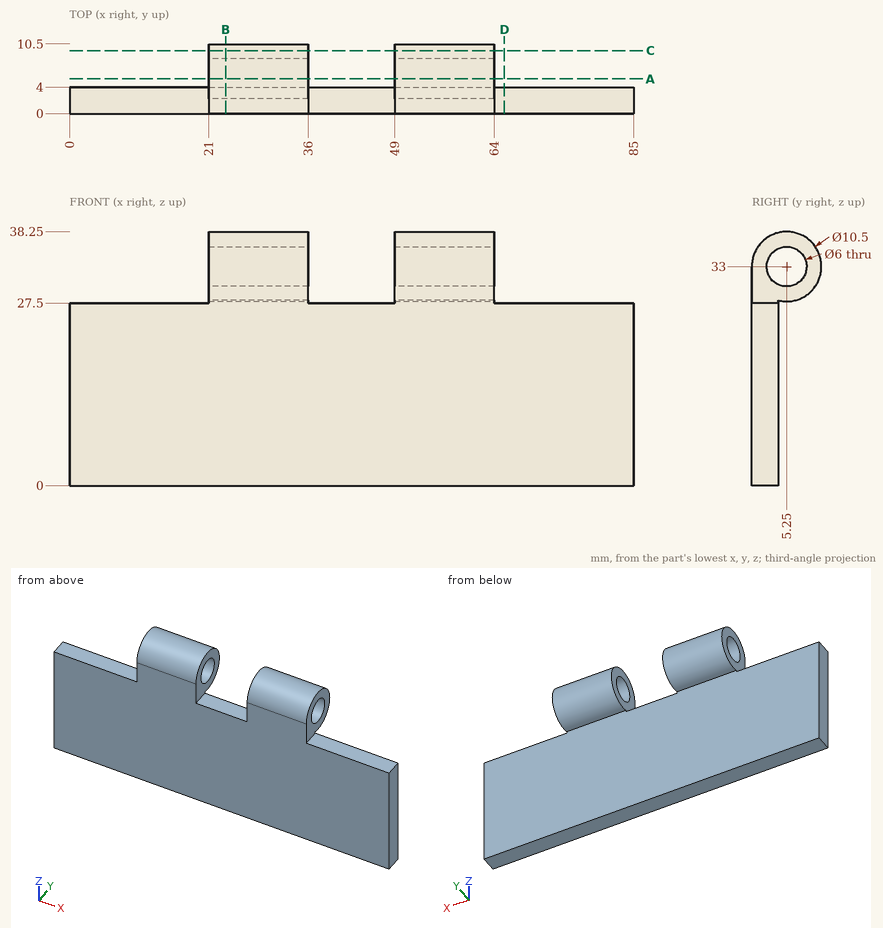
Verification items for this drawing (mm, ordinates from the low corner). Coordinates: 2 decimals unless noted, no trailing zeros. Write each loop counter-clockwise with the first axis right and the second up, starting at its lowest first coordinate (ties: lowest second). Pieces come first, ordered by that corner, then holes. Notation, with made-up numbers: (-7.5, 38.25) -> (0.5, 38.25) arc R5 cw to (0.5, 46.25) -> close; hole circle Ø6 at (46.25, 7). An arc over 180 degrees is marked (long way). One line per item, written item: value. Start each with the question number.
Q1. Cross-section at A-A on y = 5.25. Enter the section's corners in (x, z).
Q2. Cross-section at D-D on x = 65.5. Enter the section's corners in (y, z), and give its area (3 significant figures).
Q3. Cross-section at B-B on x = 23.5. Enter the section's corners in (y, z), and give its area (3 significant figures).
Q4. Go/stop test with flat-tipped pins: P1, Ø2, axis at x = 52, y = 7, coming from the +Z side; P2, Ø4.5, axis at x = 39.5, y = 1, coming from the +Z side; P3, Ø1.5, axis at x = 61, y = 9, coming from the -Z side. Record where each tip stops, or that it passes through.
Q5. Cross-section at C-C on y = 9.5. Enter the section's corners in (x, z), and give its area (3 significant figures).
Q6. Thickness scan on L1, parallel to X at y = 1.75, z = 34; L2, parallel to Y at x = 60.5, z = 33; L3, parallel to Y at x = 8.5, z = 16. Record the ranges inside material, lowest first. Write a range as from..to.
Checked values:
1. outline: (21, 27.75) -> (36, 27.75) -> (36, 30) -> (21, 30) -> close; (21, 36) -> (36, 36) -> (36, 38.25) -> (21, 38.25) -> close; (49, 27.75) -> (64, 27.75) -> (64, 30) -> (49, 30) -> close; (49, 36) -> (64, 36) -> (64, 38.25) -> (49, 38.25) -> close
2. outline: (0, 0) -> (4, 0) -> (4, 27.5) -> (0, 27.5) -> close
2. area: 110 mm²
3. outline: (0, 0) -> (4, 0) -> (4, 27.9) arc R5.25 ccw (long way) to (0, 33) -> close; hole circle Ø6 at (5.25, 33)
3. area: 175 mm²
4. P1: stops at z = 38.2
4. P2: stops at z = 27.5
4. P3: stops at z = 28.69
5. outline: (21, 29.92) -> (36, 29.92) -> (36, 36.08) -> (21, 36.08) -> close; (49, 29.92) -> (64, 29.92) -> (64, 36.08) -> (49, 36.08) -> close
5. area: 185 mm²
6. L1: x = 21..36, 49..64
6. L2: y = 0..2.25, 8.25..10.5
6. L3: y = 0..4
